Design review of the part built by this model. Coordinates are the model's own, in mm. A direction names the side the tool comes from. Give positions to 0.01 mm unless a question says otherwise; leave off trailing zeros. Loops run counter-clockwise (first coordinate to the right, second up) from the corner with the lowest first, then second, coordinate; pieces in that order, holes last. Notation, with made-up numbers: (40.25, 17) - (99.25, 17) arc R12 ccw to (99.25, 39) - close; hole circle Ø7 at (-34.5, 33.25). An arc over 180 degrees is marked (long way). One line per item, written item: value. Start each with the question number.
```python
from build123d import *

# Parameters (mm, degrees)
SKETCH1_R              = 19.5
BOSS_EXTRUDE1_DEPTH    = 185
SKETCH2_R              = 30
BOSS_EXTRUDE2_DEPTH    = 15
CHAMFER1_SIZE          = 3
CHAMFER2_SIZE          = 1
M20_TAPPED_HOLE1_D     = 17.5
M20_TAPPED_HOLE1_DEPTH = 52.5
M20_TAPPED_HOLE1_TIP   = 5.257530416


with BuildPart() as part:
    # Sketch1 → Boss-Extrude1 (new body)
    with BuildSketch(Plane.XY):
        Circle(SKETCH1_R)
    extrude(amount=BOSS_EXTRUDE1_DEPTH)

    # Sketch2 → Boss-Extrude2 (add)
    with BuildSketch(Plane.XY.offset(185)):
        Circle(SKETCH2_R)
    extrude(amount=BOSS_EXTRUDE2_DEPTH)

    # Chamfer1
    chamfer1_edges = [part.edges().sort_by_distance(p)[0] for p in [
        (-19.5, 0, 0),
    ]]
    chamfer(chamfer1_edges, length=CHAMFER1_SIZE)

    # Chamfer2
    chamfer2_edges = [part.edges().sort_by_distance(p)[0] for p in [
        (-30, 0, 185),
        (-30, 0, 200),
    ]]
    chamfer(chamfer2_edges, length=CHAMFER2_SIZE)

    # M20 Tapped Hole1
    with Locations(Plane(origin=(0, 0, 0), x_dir=(-1, 0, 0), z_dir=(0, 0, -1))):
        with Locations((0, 0)):
            Hole(M20_TAPPED_HOLE1_D / 2, depth=M20_TAPPED_HOLE1_DEPTH)
            with Locations((0, 0, -(M20_TAPPED_HOLE1_DEPTH + M20_TAPPED_HOLE1_TIP / 2))):  # 118° drill point
                Cone(0, M20_TAPPED_HOLE1_D / 2, M20_TAPPED_HOLE1_TIP, mode=Mode.SUBTRACT)


solid = part.part
```
(1) For pin 1 Ø2 at (y, z) = (9, 147.5) entering from +X; pin 2 Ø2 at (x, y) = (18, -11) entering from -Z; pin 3 Ø1 at (x, y) = (9, -17) entering from -Z, all flat-tipped, find the tip position at first contact; note any pin that passes through.
(2) To check wall thickness, follow L1, parallel to Y at x = 0, z = 18; L2, parallel to Z at x = 25, y = 8.5; L3, parallel to X at y = -2, z = 74. State the ranges of each line that lie inside material, in increasing order. Write a range as from..to.
(3) Take a section at B-B on z = 150.5. State the section outline as (x, y) points.
(4) Take a section at A-A on z = 37.5. State the section outline as (x, y) points.
(5) Draft analysis for pull direction X (two halves, no side actions). For faces 1 (the cylindrical face through (-2.539, 19.334, 92.726)), 2 (the conical face through (0.329, -1.483, 56.844)), 3 (the flat face through (0, 0, 200)), state which applies: pulls with the +X half, pulls with the -X half, needs draft (parallel to the pull), parting line crosses it, or undercut.
(6) Machinability: for faces 4 (the cylindrical face through (-29.97, 1.32, 192.41)), 5 (the cylindrical face through (-6.944, -5.324, 26.618)), which of the approach directions +Z, -Z, +X, -X, +Y, -Y give a long, thin tool a straight path to every point of the face, cutting with its end or side? Answer none if there is none.
Here are the results:
1. pin 1: x = 17.78
1. pin 2: z = 185
1. pin 3: z = 2.24
2. L1: -19.5..-8.75, 8.75..19.5
2. L2: 185..200
2. L3: -19.4..19.4
3. outline: circle Ø39 at (0, 0)
4. outline: circle Ø39 at (0, 0); hole circle Ø17.5 at (0, 0)
5. face 1: parting line crosses it
5. face 2: undercut
5. face 3: needs draft
6. face 4: +Z, -Z
6. face 5: -Z
